from build123d import *

# Parameters (mm, degrees)
SKETCH_1_R             = 10
EXTRUDE_1_DEPTH        = 415
HOLE_WIZARD_M8_1_D     = 6.8
HOLE_WIZARD_M8_1_DEPTH = 22.25
HOLE_WIZARD_M8_1_TIP   = 2.042926105
CHAMFER_1_SIZE         = 1
HOLE_WIZARD_M8_2_D     = 6.8
HOLE_WIZARD_M8_2_DEPTH = 22.25
HOLE_WIZARD_M8_2_TIP   = 2.042926105


with BuildPart() as part:
    # 草图1 → 凸台-拉伸1 (new body)
    with BuildSketch(Plane.XY):
        Circle(SKETCH_1_R)
    extrude(amount=EXTRUDE_1_DEPTH)

    # M8 螺纹孔1
    with Locations(Plane.XY.offset(415)):
        with Locations((0, 0)):
            Hole(HOLE_WIZARD_M8_1_D / 2, depth=HOLE_WIZARD_M8_1_DEPTH)
            with Locations((0, 0, -(HOLE_WIZARD_M8_1_DEPTH + HOLE_WIZARD_M8_1_TIP / 2))):  # 118° drill point
                Cone(0, HOLE_WIZARD_M8_1_D / 2, HOLE_WIZARD_M8_1_TIP, mode=Mode.SUBTRACT)

    # 倒角1
    chamfer_1_edges = [part.edges().sort_by_distance(p)[0] for p in [
        (-10, 0, 0),
        (-10, 0, 415),
    ]]
    chamfer(chamfer_1_edges, length=CHAMFER_1_SIZE)

    # M8 螺纹孔2
    with Locations(Plane(origin=(0, 0, 0), x_dir=(-1, 0, 0), z_dir=(0, 0, -1))):
        with Locations((0, 0)):
            Hole(HOLE_WIZARD_M8_2_D / 2, depth=HOLE_WIZARD_M8_2_DEPTH)
            with Locations((0, 0, -(HOLE_WIZARD_M8_2_DEPTH + HOLE_WIZARD_M8_2_TIP / 2))):  # 118° drill point
                Cone(0, HOLE_WIZARD_M8_2_D / 2, HOLE_WIZARD_M8_2_TIP, mode=Mode.SUBTRACT)


solid = part.part
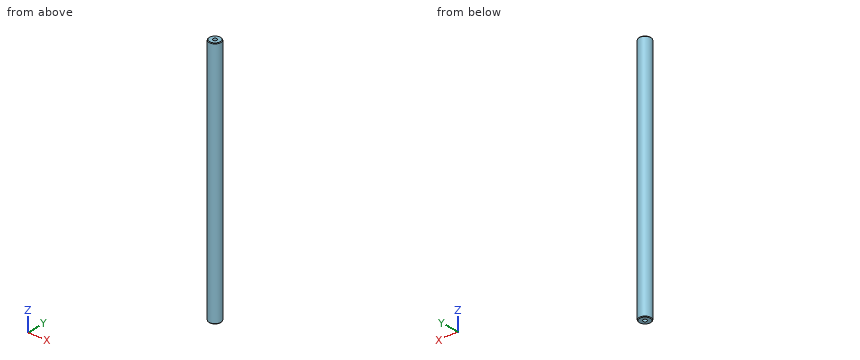
Work out the finished part from the listing and answer in its coordinate system (mm). Give positions to 0.01 mm unless a question says otherwise; leave off trailing zeros. Write each loop counter-clockwise with the first axis right and the second up, starting at its lowest first coordinate (ties: lowest second). Pieces come first, ordered by that corner, then holes. Notation, with made-up numbers: (30.25, -25) - (34.25, -25) arc R31 cw to (34.25, 14) - close; hole circle Ø11 at (72.25, 20.5). An arc over 180 degrees is marked (long way). One line per item, written item: value. Start each with the question number.
1. Consider probe 1 along Y at (x, z) = (0, 404.75); probe 2 along X at (y, z) = (4.25, 43.5); probe 3 along Z at (x, y) = (-8.5, -3). Determine where each line is inside the solid, lowest interval first.
2. Given pin 1 (3 mm diameter, centred on y = 6.5, z = 370, fed in from -X); pin 2 (5 mm diameter, centred on x = -7, z = 76, fed in from -Y); pin 3 (5 mm diameter, centred on x = -6, z = 286, fed in from +Y), each flat-ended and moving along its own axis, determine where each tip first touches the part or whether it passes through.
3. Find section A-A (z = 282.5). Write down the section's boundary in (x, y).
Geometry results:
1. probe 1: -10 to -3.4, 3.4 to 10
1. probe 2: -9.05 to 9.05
1. probe 3: 0.01 to 414.99
2. pin 1: x = -8.66
2. pin 2: y = -8.93
2. pin 3: y = 9.37
3. outline: circle Ø20 at (0, 0)
